```python
from build123d import *

# Parameters (mm, degrees)
SKETCH1_W                  = 34
SKETCH1_H                  = 110
BOSS_EXTRUDE1_DEPTH        = 6
CHAMFER1_SIZE              = 1
F_4_5_4_5_DIAMETER_HOLE1_D = 4.5
CUT_EXTRUDE1_DEPTH         = 58.879184514
SKETCH12_W                 = 14.5
SKETCH12_H                 = 60
CUT_EXTRUDE2_DEPTH         = 58.879184514
SKETCH13_W                 = 27
SKETCH13_H                 = 8
CUT_EXTRUDE3_DEPTH         = 3
FILLET1_R                  = 3
SKETCH14_R                 = 1
CUT_EXTRUDE4_DEPTH         = 3
M3_TAPPED_HOLE1_D          = 2.5
M4_TAPPED_HOLE1_D          = 3.3


with BuildPart() as part:
    # Sketch1 → Boss-Extrude1 (new body)
    with BuildSketch(Plane.XY):
        Rectangle(SKETCH1_W, SKETCH1_H)
    extrude(amount=BOSS_EXTRUDE1_DEPTH)

    # Chamfer1
    chamfer1_edges = [part.edges().sort_by_distance(p)[0] for p in [
        (-17, 55, 3),
        (17, 55, 3),
    ]]
    chamfer(chamfer1_edges, length=CHAMFER1_SIZE)

    # Ø4.5 (4.5) Diameter Hole1 (through all)
    with Locations(Plane(origin=(0, 0, 0), x_dir=(-1, 0, 0), z_dir=(0, 0, -1))):
        with Locations((-10, -50.5), (10, -50.5)):
            Hole(F_4_5_4_5_DIAMETER_HOLE1_D / 2)

    # Sketch4 → Cut-Extrude1 (cut, through all)
    with BuildSketch(Plane(origin=(0, 0, 0), x_dir=(-1, 0, 0), z_dir=(0, 0, -1))):
        with BuildLine():
            Line((-13, 44.25), (-11, 44.25))
            ThreePointArc((-11, 44.25), (-8.75, 42), (-11, 39.75))
            Line((-11, 39.75), (-13, 39.75))
            ThreePointArc((-13, 39.75), (-15.25, 42), (-13, 44.25))
        make_face()
        with BuildLine():
            Line((11, 44.25), (13, 44.25))
            ThreePointArc((13, 44.25), (15.25, 42), (13, 39.75))
            Line((13, 39.75), (11, 39.75))
            ThreePointArc((11, 39.75), (8.75, 42), (11, 44.25))
        make_face()
    extrude(amount=-CUT_EXTRUDE1_DEPTH, mode=Mode.SUBTRACT)

    # Sketch12 → Cut-Extrude2 (cut, through all)
    with BuildSketch(Plane(origin=(0, 0, 0), x_dir=(-1, 0, 0), z_dir=(0, 0, -1))):
        Rectangle(SKETCH12_W, SKETCH12_H)
    extrude(amount=-CUT_EXTRUDE2_DEPTH, mode=Mode.SUBTRACT)

    # Sketch13 → Cut-Extrude3 (cut)
    with BuildSketch(Plane(origin=(0, 0, 0), x_dir=(-1, 0, 0), z_dir=(0, 0, -1))):
        with Locations((0, -6)):
            Rectangle(SKETCH13_W, SKETCH13_H)
    extrude(amount=-CUT_EXTRUDE3_DEPTH, mode=Mode.SUBTRACT)

    # Fillet1
    fillet1_edges = [part.edges().sort_by_distance(p)[0] for p in [
        (-7.25, 30, 3),
        (-7.25, -30, 3),
        (7.25, -30, 3),
        (7.25, 30, 3),
    ]]
    fillet(fillet1_edges, radius=FILLET1_R)

    # Sketch14 → Cut-Extrude4 (cut)
    with BuildSketch(Plane(origin=(0, 0, 0), x_dir=(-1, 0, 0), z_dir=(0, 0, -1))):
        with Locations((-13.5, -2)):
            Circle(SKETCH14_R)
        with Locations((-13.5, -10)):
            Circle(SKETCH14_R)
        with Locations((13.5, -10)):
            Circle(SKETCH14_R)
        with Locations((13.5, -2)):
            Circle(SKETCH14_R)
    extrude(amount=-CUT_EXTRUDE4_DEPTH, mode=Mode.SUBTRACT)

    # M3 Tapped Hole1 (through all)
    with Locations(Plane(origin=(0, 0, 0), x_dir=(-1, 0, 0), z_dir=(0, 0, -1))):
        with Locations((-10, -6), (10, -6)):
            Hole(M3_TAPPED_HOLE1_D / 2)

    # M4 Tapped Hole1 (through all)
    with Locations(Plane.XY.offset(6)):
        with Locations((0, -39)):
            Hole(M4_TAPPED_HOLE1_D / 2)


solid = part.part
```
Geometry: final body of the model. Coordinates: model frame, mm. A direction names the side the tool comes from. Round coordinates to 2 decimals unless told otherwise and drop trailing zeros. Write each loop counter-clockwise with the first axis right and the second up, starting at its lowest first coordinate (ties: lowest second). Pieces come first, ordered by that corner, then holes. Notation, with made-up numbers: M 7.25,10 L 49.25,10 A14 ccw 49.25,37 Z; hole C 56.25,82.25 d4. An arc over 180 degrees is marked long. Answer in a Markdown table with one row per item. Add a question column.
(1) Contact query for a flat-ended pin moving along its axis: pin 1 (1.2 mm diameter, centred on x = -13.5, y = -2, fed in from -Z). Output: stop coordinate, or through.
(2) Draft query along X for faces 4 (the face through (17, -1, 3)), 5 (the face through (14.183, -1.27, 1.479)), 6 (the face through (-8, 1, 0)). Return one class per face: pulls with the +X half, pulls with the -X half, needs draft (parallel to the pull), parting line crosses it, or undercut.
(3) Reachability of faces 1 (the face through (-12, 44.25, 3)), 2 (the face through (-17, -1, 3)), 3 (the face through (-10, -2, 1)) from +Z, -Z, +X, -X, +Y, -Y: full face, straight path, thin tool, end or side. Return the list, or none.
(4) Cut plane A-A, the plane x = 3. Return the cut outline in (y, z).
(5) Ray query, L1, parallel to X at y = 16.5, z = 1.75; L2, parallel to Y at x = 14, z = 1.6; L3, parallel to Y at x = 13, z = 5.05. Return the intervals inside material, ascending.
(6) Cut plane B-B, the plane x = -10. Return the cut outline in (y, z).
(7) Cut plane C-C, the plane z = 4.65. Give the number of separate pieces and of enclosed holes in the cut face, then the cut area to 3 significant figures.
Established:
| question | item | result |
|---|---|---|
| 1 | pin 1 | z = 3 |
| 2 | face 4 | pulls with the +X half |
| 2 | face 5 | undercut |
| 2 | face 6 | needs draft |
| 3 | face 1 | +Z, -Z |
| 3 | face 2 | +Z, -Z, -X, +Y, -Y |
| 3 | face 3 | -Z |
| 4 | outline | M -55,0 L -30,0 L -30,6 L -55,6 Z; M 30,0 L 55,0 L 55,6 L 30,6 Z |
| 5 | L1 | -17 to -7.25, 7.25 to 17 |
| 5 | L2 | -55 to -10.87, -9.13 to -2.87, -1.13 to 39.98, 44.02 to 55 |
| 5 | L3 | -55 to 39.75, 44.25 to 55 |
| 6 | outline | M -55,0 L -52.75,0 L -52.75,6 L -55,6 Z; M -48.25,0 L -10,0 L -10,3 L -7.25,3 L -7.25,6 L -48.25,6 Z; M -4.75,3 L -2,3 L -2,0 L 39.98,0 L 39.98,6 L -4.75,6 Z; M 44.02,0 L 55,0 L 55,6 L 44.02,6 Z |
| 7 | separate pieces | 1 |
| 7 | enclosed holes | 8 |
| 7 | area | 2,780 mm² |
